from build123d import *
from build123d.topology import SkipClean

# Parameters (mm, degrees)
BASE_FLANGE_SKETCH_R               = 100
BASE_FLANGE_200_DEPTH              = 30
MOUNTING_PAD_DEPTH                 = 28
MOUNTING_COUNTERBORES_SKETCH_R     = 7
MOUNTING_COUNTERBORES_4X_14_DEPTH  = 8
MOUNTING_HOLES_SKETCH_R            = 4.25
MOUNTING_HOLES_4X_8_5_DEPTH        = 50
SUPPORT_BOSS_DEPTH                 = 42
BEARING_COUNTERBORE_SKETCH_R       = 20
BEARING_COUNTERBORE_40_DEPTH       = 8
BEARING_BORE_SKETCH_R              = 12.5
BEARING_BORE_25_DEPTH              = 30
THROUGH_BORE_SKETCH_R              = 5
THROUGH_BORE_10_DEPTH              = 13
UNDERSIDE_RECESS_SKETCH_R          = 40
UNDERSIDE_RECESS_80_DEPTH          = 25
SIDE_SLOT_DEPTH                    = 14
BOSS_HOLE_COUNTERBORES_SKETCH_R    = 5
BOSS_HOLE_COUNTERBORES_2X_10_DEPTH = 8
BOSS_PIN_HOLES_SKETCH_R            = 3
BOSS_PIN_HOLES_2X_6_DEPTH          = 23.8


with BuildPart() as part:
    # Base Flange Sketch → Base Flange Ø200 (new body)
    with BuildSketch(Plane(origin=(0, 0, 0), x_dir=(1, 0, 0), z_dir=(0, 1, 0))):
        with Locations(Location((0, 0, 0), (0, 0, 270))):
            Circle(BASE_FLANGE_SKETCH_R)
    extrude(amount=BASE_FLANGE_200_DEPTH)

    # Mounting Pad Sketch → Mounting Pad (add)
    with SkipClean():  # the faces are left unmerged after this step: merging them gives an invalid solid
        with BuildSketch(Plane(origin=(0, 30, 0), x_dir=(1, 0, 0), z_dir=(0, 1, 0))):
            with BuildLine():
                Line((68.053287944, 25), (96.824583655, 25))
                ThreePointArc((96.824583655, 25), (100, 0), (96.824583655, -25))
                Line((96.824583655, -25), (68.053287944, -25))
                ThreePointArc((68.053287944, -25), (51.265241636, -51.265241636), (25, -68.053287944))
                Line((25, -68.053287944), (25, -96.824583655))
                ThreePointArc((25, -96.824583655), (0, -100), (-25, -96.824583655))
                Line((-25, -96.824583655), (-25, -68.053287944))
                ThreePointArc((-25, -68.053287944), (-51.265241636, -51.265241636), (-68.053287944, -25))
                Line((-68.053287944, -25), (-96.824583655, -25))
                ThreePointArc((-96.824583655, -25), (-100, 0), (-96.824583655, 25))
                Line((-96.824583655, 25), (-68.053287944, 25))
                ThreePointArc((-68.053287944, 25), (-51.265241636, 51.265241636), (-25, 68.053287944))
                Line((-25, 68.053287944), (-25, 96.824583655))
                ThreePointArc((-25, 96.824583655), (0, 100), (25, 96.824583655))
                Line((25, 96.824583655), (25, 68.053287944))
                ThreePointArc((25, 68.053287944), (51.265241636, 51.265241636), (68.053287944, 25))
            make_face()
        extrude(amount=MOUNTING_PAD_DEPTH)

    # Mounting Counterbores Sketch → Mounting Counterbores 4xØ14 (cut)
    with SkipClean():  # the faces are left unmerged after this step: merging them gives an invalid solid
        with BuildSketch(Plane(origin=(0, 58, 0), x_dir=(1, 0, 0), z_dir=(0, 1, 0))):
            with Locations(Location((0, 84.5, 0), (0, 0, 270))):
                Circle(MOUNTING_COUNTERBORES_SKETCH_R)
            with Locations(Location((84.5, 0, 0), (0, 0, 270))):
                Circle(MOUNTING_COUNTERBORES_SKETCH_R)
            with Locations(Location((0, -84.5, 0), (0, 0, 270))):
                Circle(MOUNTING_COUNTERBORES_SKETCH_R)
            with Locations(Location((-84.5, 0, 0), (0, 0, 270))):
                Circle(MOUNTING_COUNTERBORES_SKETCH_R)
        extrude(amount=-MOUNTING_COUNTERBORES_4X_14_DEPTH, mode=Mode.SUBTRACT)

    # Mounting Holes Sketch → Mounting Holes 4xØ8.5 (cut)
    with SkipClean():  # the faces are left unmerged after this step: merging them gives an invalid solid
        with BuildSketch(Plane(origin=(0, 50, 0), x_dir=(1, 0, 0), z_dir=(0, 1, 0))):
            with Locations(Location((0, 84.5, 0), (0, 0, 270))):
                Circle(MOUNTING_HOLES_SKETCH_R)
            with Locations(Location((84.5, 0, 0), (0, 0, 270))):
                Circle(MOUNTING_HOLES_SKETCH_R)
            with Locations(Location((0, -84.5, 0), (0, 0, 270))):
                Circle(MOUNTING_HOLES_SKETCH_R)
            with Locations(Location((-84.5, 0, 0), (0, 0, 270))):
                Circle(MOUNTING_HOLES_SKETCH_R)
        extrude(amount=-MOUNTING_HOLES_4X_8_5_DEPTH, mode=Mode.SUBTRACT)

    # Support Boss Sketch → Support Boss (add)
    with SkipClean():  # the faces are left unmerged after this step: merging them gives an invalid solid
        with BuildSketch(Plane(origin=(0, 58, 0), x_dir=(1, 0, 0), z_dir=(0, 1, 0))):
            with BuildLine():
                Line((-6.670404666, 52.671203723), (-23.359173661, 8.907805895))
                ThreePointArc((-23.359173661, 8.907805895), (-24.999857744, 0.084337338), (-23.418742494, -8.75))
                Line((-23.418742494, -8.75), (-7.025622749, -52.625))
                ThreePointArc((-7.025622749, -52.625), (-1e-09, -57.5), (7.025622747, -52.625))
                Line((7.025622747, -52.625), (23.418742494, -8.75))
                ThreePointArc((23.418742494, -8.75), (24.999857744, -0.084337338), (23.477245263, 8.591795789))
                Line((23.477245263, 8.591795789), (7.380521011, 52.576400691))
                ThreePointArc((7.380521011, 52.576400691), (0.387949547, 57.498691247), (-6.670404666, 52.671203723))
            make_face()
        extrude(amount=SUPPORT_BOSS_DEPTH)

    # Bearing Counterbore Sketch → Bearing Counterbore Ø40 (cut)
    with SkipClean():  # the faces are left unmerged after this step: merging them gives an invalid solid
        with BuildSketch(Plane(origin=(0, 100, 0), x_dir=(1, 0, 0), z_dir=(0, 1, 0))):
            with Locations(Location((0, 0, 0), (0, 0, 270))):
                Circle(BEARING_COUNTERBORE_SKETCH_R)
        extrude(amount=-BEARING_COUNTERBORE_40_DEPTH, mode=Mode.SUBTRACT)

    # Bearing Bore Sketch → Bearing Bore Ø25 (cut)
    with SkipClean():  # the faces are left unmerged after this step: merging them gives an invalid solid
        with BuildSketch(Plane(origin=(0, 92, 0), x_dir=(1, 0, 0), z_dir=(0, 1, 0))):
            with Locations(Location((0, 0, 0), (0, 0, 270))):
                Circle(BEARING_BORE_SKETCH_R)
        extrude(amount=-BEARING_BORE_25_DEPTH, mode=Mode.SUBTRACT)

    # Through Bore Sketch → Through Bore Ø10 (cut)
    with SkipClean():  # the faces are left unmerged after this step: merging them gives an invalid solid
        with BuildSketch(Plane(origin=(0, 62, 0), x_dir=(1, 0, 0), z_dir=(0, 1, 0))):
            with Locations(Location((0, 0, 0), (0, 0, 270))):
                Circle(THROUGH_BORE_SKETCH_R)
        extrude(amount=-THROUGH_BORE_10_DEPTH, mode=Mode.SUBTRACT)

    # Underside Recess Sketch → Underside Recess Ø80 (cut)
    with SkipClean():  # the faces are left unmerged after this step: merging them gives an invalid solid
        with BuildSketch(Plane.XZ):
            with Locations(Location((0, 0, 0), (0, 0, 270))):
                Circle(UNDERSIDE_RECESS_SKETCH_R)
        extrude(amount=-UNDERSIDE_RECESS_80_DEPTH, mode=Mode.SUBTRACT)

    # Side Slot Sketch → Side Slot (cut, symmetric)
    with SkipClean():  # the faces are left unmerged after this step: merging them gives an invalid solid
        with BuildSketch(Plane(origin=(0, 0, 0), x_dir=(0, 0, -1), z_dir=(1, 0, 0))):
            with BuildLine():
                Line((-28, 25), (28, 25))
                Line((28, 25), (28, 39.42))
                ThreePointArc((28, 39.42), (25.194082964, 46.194082964), (18.42, 49))
                Line((18.42, 49), (-18.42, 49))
                ThreePointArc((-18.42, 49), (-25.194082964, 46.194082964), (-28, 39.42))
                Line((-28, 39.42), (-28, 25))
            make_face()
        extrude(amount=SIDE_SLOT_DEPTH, both=True, mode=Mode.SUBTRACT)

    # Boss Hole Counterbores Sketch → Boss Hole Counterbores 2xØ10 (cut)
    with SkipClean():  # the faces are left unmerged after this step: merging them gives an invalid solid
        with BuildSketch(Plane(origin=(0, 100, 0), x_dir=(1, 0, 0), z_dir=(0, 1, 0))):
            with Locations(Location((0.337347432, 49.998861954, 0), (0, 0, 270))):
                Circle(BOSS_HOLE_COUNTERBORES_SKETCH_R)
            with Locations(Location((-1e-09, -50, 0), (0, 0, 270))):
                Circle(BOSS_HOLE_COUNTERBORES_SKETCH_R)
        extrude(amount=-BOSS_HOLE_COUNTERBORES_2X_10_DEPTH, mode=Mode.SUBTRACT)

    # Boss Pin Holes Sketch → Boss Pin Holes 2xØ6 (cut)
    with SkipClean():  # the faces are left unmerged after this step: merging them gives an invalid solid
        with BuildSketch(Plane(origin=(0, 92, 0), x_dir=(1, 0, 0), z_dir=(0, 1, 0))):
            with Locations(Location((0.337347432, 49.998861954, 0), (0, 0, 270))):
                Circle(BOSS_PIN_HOLES_SKETCH_R)
            with Locations(Location((-1e-09, -50, 0), (0, 0, 270))):
                Circle(BOSS_PIN_HOLES_SKETCH_R)
        extrude(amount=-BOSS_PIN_HOLES_2X_6_DEPTH, mode=Mode.SUBTRACT)


solid = part.part
The listing builds one solid part. Answer for the finished solid, in the listing's coordinates (mm). A direction names the side the tool comes from. Round coordinates to 2 decimals unless told otherwise and drop trailing zeros. Write each loop counter-clockwise with the first axis right and the second up, starting at its lowest first coordinate (ties: lowest second). Pieces come first, ordered by that corner, then holes. Notation, with made-up numbers: M 82.25,43 L 125.25,43 A7 ccw 125.25,56 Z; hole C 7,4 d8. An arc over 180 degrees is marked long. Write each question's results on one line, items separated by ' | '. Start each with the question number.
(1) Each of these flat-tipped pins is pushed along its axis until it touches: P1, Ø5, axis at x = -53, z = -36.5, coming from the +Y side; P2, Ø6, axis at y = 11.5, z = -29, coming from the +X side; P3, Ø11, axis at x = 84.5, z = -0.5, coming from the +Y side. Where does it stop, or does it pass through?
(2) The part is cut by section D-D, the plane x = 60.5. Write down the section's boundary in (y, z).
(3) The part is cut by section A-A, the plane y = 12.5. Write down the section's boundary in (x, z), and give its area (3 significant figures).
(4) The part is cut by section C-C, the plane z = -84.5. Write down the section's boundary in (x, y), and give its area (3 significant figures).
(5) For faces 5 (the cylindrical face through (-39.05, 12.32, 8.67)), 6 (the flat face through (-88, 50, 3)), 7 (the flat face through (-25, 44, 83)), 8 (the cylindrical face through (25, 79, 0)), determine the directions among +Z, -Z, +X, -X, +Y, -Y from which every point of the face is accessible in a straight line to the end or side of a thin tool.
(6) Find the intervals of material crossed by line 1 (X direction, y = 53.5, z = 0); line 2 (X direction, y = 97.5, z = 0); line 3 (X direction, y = 35, z = 84.5), in increasing order.
(7) The part is cut by section B-B, the plane x = 84.5. Write down the section's boundary in (y, z).
(8) Determine the mould class of faces 1 (the cylindrical face through (91.44, 54.06, -0.91)), 2 (the cylindrical face through (-25, 79, 0)), 3 (the flat face through (61, 30, 60)), 4 (the flat face through (82, 44, -25)) for opening direction Z: +Z half, -Z half, draft (parallel to the pull), parting line (faces both ways), or undercut.
Worked answers:
1) P1: stops at y = 58 | P2: stops at x = 96.56 | P3: stops at y = 50
2) outline: M 0,-79.62 L 30,-79.62 L 30,-39.95 L 58,-39.95 L 58,39.95 L 30,39.95 L 30,79.62 L 0,79.62 Z
3) outline: C 0,0 d200; hole C -84.5,0 d8.5; hole C 0,0 d80; hole C 0,-84.5 d8.5; hole C 0,84.5 d8.5; hole C 84.5,0 d8.5 | area: 26,200 mm²
4) outline: M -53.48,0 L -4.25,0 L -4.25,50 L -7,50 L -7,58 L -25,58 L -25,30 L -53.48,30 Z; M 4.25,0 L 53.48,0 L 53.48,30 L 25,30 L 25,58 L 7,58 L 7,50 L 4.25,50 Z | area: 4,070 mm²
5) face 5: -Y | face 6: +Y | face 7: +Z, -X, +Y | face 8: +X, +Y
6) line 1: x = -100 to -91.5, -77.5 to -5, 5 to 77.5, 91.5 to 100 | line 2: x = -25 to -20, 20 to 25 | line 3: x = -25 to -4.25, 4.25 to 25
7) outline: M 0,-53.48 L 30,-53.48 L 30,-25 L 58,-25 L 58,-7 L 50,-7 L 50,-4.25 L 0,-4.25 Z; M 0,4.25 L 50,4.25 L 50,7 L 58,7 L 58,25 L 30,25 L 30,53.48 L 0,53.48 Z
8) face 1: undercut | face 2: parting line | face 3: draft | face 4: -Z half
